Here's the drawing with two shaded views (mm, measured from the low corner). I have some questions. A direction names the side the tool comes from. Give positions to 0.01 mm unless a question says otherwise; leave off trailing zeros. Loops run counter-clockwise (first coordinate to the right, second up) from the corner with the lowest first, then second, coordinate; pieces in that order, holes last. Notation, with made-up numbers: M 71,-13.75 L 94,-13.75 A9 ccw 94,-4.75 Z; hole C 24,33.5 d9. An arc over 180 degrees is marked long. Use a Markdown table: item, result. Add a question column.
1) Suppose I cut it at A-A on x = 7.5. List the corners of the cut face in (y, z) for me.
2) Suppose I cut it at B-B on y = 0.8. List the corners of the cut face in (x, z) for me, and give its area (3 significant figures).
3) We'd pull the mould along Y, two halves only. Please class the marked faces 6, 7, 8 and 9: +Y half, -Y half, draft (parallel to the pull), parting line (faces both ways), or undercut.
4) Suppose I cut it at C-C on x = 2.75. List the corners of the cut face in (y, z) for me.
5) Will these pins go through, and if not, where does the flat tip stop? pin 1 Ø1.5 at (x, z) = (1.5, 3.5) entering from +Y; pin 2 Ø1 at (x, y) = (1, 3.5) entering from -Z; pin 3 Ø2.5 at (y, z) = (4, 1.5) entering from -X; pin 4 Ø1.8 at (x, y) = (5.5, 3.5) entering from -Z.
6) Which directions (+Z, -Z, +X, -X, +Y, -Y) give clear straight access to the entire face, cutting with the end or side of a thin tool? Please do the marked faces 1, 2, 3, 4 and 5.
7) If I drill on line 1 along Y through (x, z) = (3.7, 1.5); line 2 along Y through (x, z) = (3.3, 1.5); line 3 along Y through (x, z) = (6, 5.5), over which ranges is the centre line in solid material (lowest first)? Write a range as [from, to].
8) Suppose I cut it at D-D on z = 1.15. List the corners of the cut face in (x, y) for me.
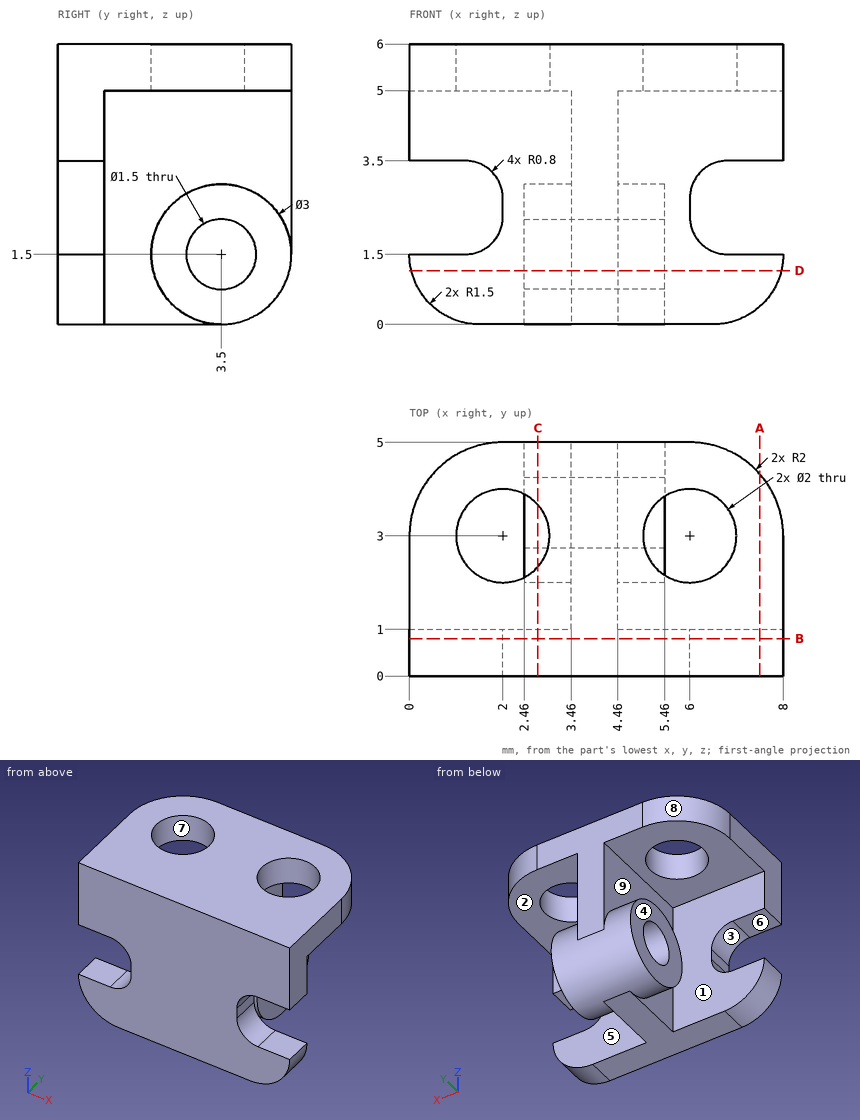
Answer block:
| question | item | result |
|---|---|---|
| 1 | outline | M 0,0.38 L 1,0.38 L 1,1.5 L 0,1.5 Z; M 0,3.5 L 1,3.5 L 1,5 L 4.32,5 L 4.32,6 L 0,6 Z |
| 2 | outline | M 0,1.5 A1.5 ccw 1.5,0 L 6.5,0 A1.5 ccw 8,1.5 L 6.8,1.5 A0.8 cw 6,2.3 L 6,2.7 A0.8 cw 6.8,3.5 L 8,3.5 L 8,6 L 0,6 L 0,3.5 L 1.2,3.5 A0.8 cw 2,2.7 L 2,2.3 A0.8 cw 1.2,1.5 Z |
| 2 | area | 39.6 mm^2 |
| 3 | face 6 | draft |
| 3 | face 7 | undercut |
| 3 | face 8 | +Y half |
| 3 | face 9 | undercut |
| 4 | outline | M 0,0 L 1,0 L 1,5 L 2.34,5 L 2.34,6 L 0,6 Z; C 3.5,1.5 d3; M 3.66,5 L 5,5 L 5,6 L 3.66,6 Z; hole C 3.5,1.5 d1.5 |
| 5 | pin 1 | stops at y = 1 |
| 5 | pin 2 | stops at z = 5 |
| 5 | pin 3 | stops at x = 2.46 |
| 5 | pin 4 | stops at z = 0 |
| 6 | face 1 | -Z, -X |
| 6 | face 2 | +X, +Y |
| 6 | face 3 | -X, +Y, -Y |
| 6 | face 4 | -Z, -X, +Y |
| 6 | face 5 | -Z, +X |
| 7 | line 1 | y = [0, 2.75], [4.25, 5] |
| 7 | line 2 | y = [0, 1], [2, 2.75], [4.25, 5] |
| 7 | line 3 | y = [0, 2], [4, 5] |
| 8 | outline | M 0.04,0 L 7.96,0 L 7.96,1 L 4.46,1 L 4.46,2.04 L 5.46,2.04 L 5.46,2.84 L 2.46,2.84 L 2.46,2.04 L 3.46,2.04 L 3.46,1 L 0.04,1 Z; M 2.46,4.16 L 5.46,4.16 L 5.46,4.96 L 2.46,4.96 Z |
